Design review of the part built by this model. Coordinates are the model's own, in mm. Face numbers are marked on the shaded views. A direction names the side the tool comes from. Round coordinates to 2 decimals unless told otherwise and drop trailing zeros. Loops run counter-clockwise (first coordinate to the right, second up) from the corner with the lowest first, then second, coordinate; pieces in that order, holes last. Notation, with made-up numbers: (0.25, 60) - (16.25, 60) arc R12 cw to (16.25, 72) - close; hole circle Ø6 at (44.25, 70.5). An arc over 180 degrees is marked (long way). Answer as CSV lines item,"result". Start each with the question number.
(1) Consider section C-C (z = 13). Give the boundary of the cut face in (x, y), and give its area (3 significant figures).
(2) For P1, Ø6, axis at x = 45, z = 5.5, coming from the -Y side; P2, Ø12, axis at y = 23, z = -12.5, coming from the -X side; P3, Ø2, axis at y = 10, z = 1, coming from the +X side, all flat-tipped, find the tip position at first contact; note any pin that passes through.
(3) Consider section D-D (y = 25.5). Give the boundary of the cut face in (x, z), and give its area (3 significant figures).
(4) Consider section A-A (y = 18.75). Give the boundary of the cut face in (x, z).
(5) Consider section B-B (y = 5). Give the boundary of the cut face in (x, z).
(6) Mouldability with a two-part tool opening along X and no side actions: class the marked faces 6, 7 and 8 as released by +X, released by -X, zero draft, split by the parting line, or undercut.
(7) Wall thickness on L1, parallel to Z at x = 61, y = 24; L2, parallel to Y at x = 32, z = -8.5; L3, parallel to Y at x = -2, z = 12.5: over which ranges is each line inside the solid? List them lowest first.
(8) For the marked faces 1, 2, 3, 4 and 5, list the 3-axis set-ups (+Z, -Z, +X, -X, +Y, -Y) from which the entire face can be reached by the end or side of a thin tool; tool diameter is ignored.
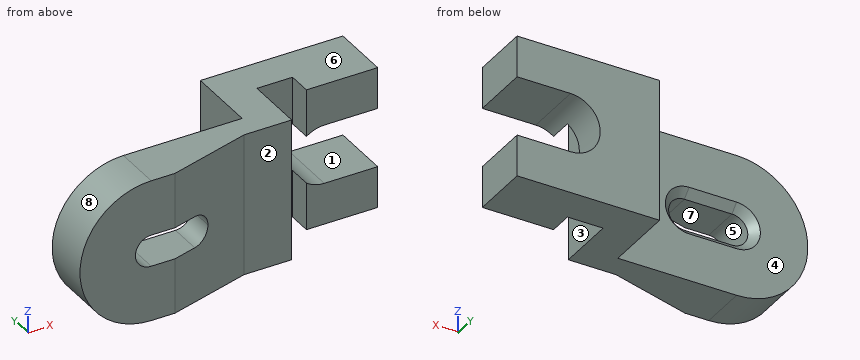
from build123d import *

# Parameters (mm, degrees)
HUB_SKETCH_R                = 18
HUB_36_DEPTH                = 12
ARM_START                   = -12
ARM_DEPTH                   = 12
HUB_SLOT_CHAMFER_45_DEPTH   = 2
HUB_SLOT_CHAMFER_45_DRAFT   = -45
HUB_SLOT_DEPTH              = 18
CLEVIS_BLOCK_DEPTH          = 36
CLEVIS_U_SLOT_SKETCH_W      = 13.5
CLEVIS_U_SLOT_SKETCH_H      = 15
CLEVIS_U_SLOT_DEPTH         = 90
BLOCK_STEP_CUT_DEPTH        = 60
BLOCK_STEP_CUT_DEPTH_BACK   = 147
BLOCK_STEP_CUT_SKETCH_W     = 9
BLOCK_STEP_CUT_SKETCH_H     = 21
ARM_TAPER_CUT_DEPTH         = 73
ARM_TAPER_CUT_DEPTH_BACK    = 190
ARM_TAPER_CUT_SKETCH_W      = 18
ARM_TAPER_CUT_SKETCH_H      = 15
BLOCK_RELIEF_CUT_DEPTH      = 190
BLOCK_RELIEF_CUT_DEPTH_BACK = 190


with BuildPart() as part:
    # Hub Sketch → Hub _36 (new body)
    with BuildSketch(Plane(origin=(0, 0, 0), x_dir=(1, 0, 0), z_dir=(0, 1, 0))):
        with Locations(Location((0, 0, 0), (0, 0, 270))):
            Circle(HUB_SKETCH_R)
    extrude(amount=HUB_36_DEPTH)

    # Arm Sketch → Arm (add)
    with BuildSketch(Plane(origin=(0, 12, 0), x_dir=(1, 0, 0), z_dir=(0, 1, 0)).offset(ARM_START)):
        with BuildLine():
            Line((30, 0), (18, 0))
            ThreePointArc((18, 0), (12.727922061, -12.727922061), (0, -18))
            Line((0, -18), (30, -18))
            Line((30, -18), (30, 0))
        make_face()
        with BuildLine():
            ThreePointArc((0, 18), (12.727922061, 12.727922061), (18, 0))
            Line((18, 0), (30, 0))
            Line((30, 0), (30, 18))
            Line((30, 18), (0, 18))
        make_face()
    extrude(amount=ARM_DEPTH)


with BuildPart() as hub_slot_chamfer_45_tool:
    # Hub Slot Chamfer Sketch → Hub Slot Chamfer 45 (with draft: the straight prism first)
    with BuildSketch(Plane(origin=(0, 12, 0), x_dir=(1, 0, 0), z_dir=(0, 1, 0))):
        with BuildLine():
            ThreePointArc((0, 6), (-6, 0), (0, -6))
            Line((0, -6), (12, -6))
            ThreePointArc((12, -6), (18, 0), (12, 6))
            Line((12, 6), (0, 6))
        make_face()
    extrude(amount=-HUB_SLOT_CHAMFER_45_DEPTH)
    # Hub Slot Chamfer 45: the draft: its side faces are tilted about the plane it starts from
    hub_slot_chamfer_45_sides = [hub_slot_chamfer_45_tool.faces().sort_by_distance(p)[0] for p in [
        (6, 11, -6),
        (-6, 11, 0),
        (6, 11, 6),
        (18, 11, 0),
    ]]
    draft(hub_slot_chamfer_45_sides, Plane(origin=(0, 12, 0), x_dir=(1, 0, 0), z_dir=(0, 1, 0)), HUB_SLOT_CHAMFER_45_DRAFT)


with BuildPart() as part_1:
    add(part.part)

    # Hub Slot Chamfer 45: cut by hub_slot_chamfer_45_tool
    add(hub_slot_chamfer_45_tool.part, mode=Mode.SUBTRACT)

    # Hub Slot Sketch → Hub Slot (cut)
    with BuildSketch(Plane(origin=(0, 10, 0), x_dir=(1, 0, 0), z_dir=(0, 1, 0))):
        with BuildLine():
            Line((12, 4), (0, 4))
            ThreePointArc((0, 4), (2.828427125, 2.828427125), (4, 0))
            ThreePointArc((4, 0), (2.828427125, -2.828427125), (0, -4))
            Line((0, -4), (12, -4))
            ThreePointArc((12, -4), (8, 0), (12, 4))
        make_face()
        with BuildLine():
            ThreePointArc((4, 0), (2.828427125, 2.828427125), (0, 4))
            ThreePointArc((0, 4), (-4, 0), (0, -4))
            ThreePointArc((0, -4), (2.828427125, -2.828427125), (4, 0))
        make_face()
        with BuildLine():
            ThreePointArc((16, 0), (14.828427125, 2.828427125), (12, 4))
            ThreePointArc((12, 4), (8, 0), (12, -4))
            ThreePointArc((12, -4), (14.828427125, -2.828427125), (16, 0))
        make_face()
    extrude(amount=-HUB_SLOT_DEPTH, mode=Mode.SUBTRACT)

    # Clevis Block Sketch → Clevis Block (add)
    with BuildSketch(Plane.XY.offset(18)):
        Polygon((30, 12), (30, 30), (66, 30), (66, 15), (66, 0), (30, 0), align=None)
    extrude(amount=-CLEVIS_BLOCK_DEPTH)

    # Clevis U-Slot Sketch → Clevis U-Slot (cut)
    with BuildSketch(Plane(origin=(0, 30, 0), x_dir=(1, 0, 0), z_dir=(0, 1, 0))):
        with BuildLine():
            Line((52.5, -7.5), (52.5, 7.5))
            ThreePointArc((52.5, 7.5), (45, 0), (52.5, -7.5))
        make_face()
        with Locations((59.25, 0)):
            Rectangle(CLEVIS_U_SLOT_SKETCH_W, CLEVIS_U_SLOT_SKETCH_H)
    extrude(amount=-CLEVIS_U_SLOT_DEPTH, mode=Mode.SUBTRACT)

    # Block Step Cut Sketch → Block Step Cut (cut, two sides: drawn at the far end of the back side and taken through both)
    with BuildSketch(Plane.XY.offset(18).offset(-BLOCK_STEP_CUT_DEPTH_BACK)):
        with Locations((43.5, 10.5)):
            Rectangle(BLOCK_STEP_CUT_SKETCH_W, BLOCK_STEP_CUT_SKETCH_H)
    extrude(amount=BLOCK_STEP_CUT_DEPTH + BLOCK_STEP_CUT_DEPTH_BACK, mode=Mode.SUBTRACT)

    # Arm Taper Cut Sketch → Arm Taper Cut (cut, two sides: drawn at the far end of the back side and taken through both)
    with BuildSketch(Plane.XY.offset(18).offset(-ARM_TAPER_CUT_DEPTH_BACK)):
        with Locations((57, 7.5)):
            Rectangle(ARM_TAPER_CUT_SKETCH_W, ARM_TAPER_CUT_SKETCH_H)
    extrude(amount=ARM_TAPER_CUT_DEPTH + ARM_TAPER_CUT_DEPTH_BACK, mode=Mode.SUBTRACT)

    # Block Relief Cut Sketch → Block Relief Cut (cut, two sides: drawn at the far end of the back side and taken through both)
    with BuildSketch(Plane.XY.offset(18).offset(-BLOCK_RELIEF_CUT_DEPTH_BACK)):
        Polygon((39, 0), (39, 6), (27, 6), (6, 0), align=None)
    extrude(amount=BLOCK_RELIEF_CUT_DEPTH + BLOCK_RELIEF_CUT_DEPTH_BACK, mode=Mode.SUBTRACT)


solid = part_1.part
Determined:
1,outline,"(-12.45, 0) - (6, 0) - (27, 6) - (39, 6) - (39, 21) - (48, 21) - (48, 15) - (66, 15) - (66, 30) - (30, 30) - (30, 12) - (-12.45, 12) - close"
1,area,"995 mm^2"
2,P1,"stops at y = 21"
2,P2,"stops at x = 30"
2,P3,"stops at x = 39"
3,outline,"(30, -18) - (66, -18) - (66, -7.5) - (52.5, -7.5) arc R7.5 cw to (52.5, 7.5) - (66, 7.5) - (66, 18) - (30, 18) - close"
3,area,"1,010 mm^2"
4,outline,"(30, -18) - (39, -18) - (39, 18) - (30, 18) - close; (48, -18) - (66, -18) - (66, -7.5) - (52.5, -7.5) arc R7.5 cw to (48, -6) - close; (48, 6) arc R7.5 cw to (52.5, 7.5) - (66, 7.5) - (66, 18) - (48, 18) - close"
5,outline,"(0, -18) - (23.5, -18) - (23.5, 18) - (0, 18) arc R18 ccw to start; hole (0, -4) - (12, -4) arc R4 ccw to (12, 4) - (0, 4) arc R4 ccw to start"
6,face 6,"zero draft"
6,face 7,"undercut"
6,face 8,"released by -X"
7,L1,"z = -18 to -7.5, 7.5 to 18"
7,L2,"y = 6 to 30"
7,L3,"y = 0 to 12"
8,face 1,"+X, +Y, -Y"
8,face 2,"+Z, -Z, +X, -Y"
8,face 3,"+Z, -Z, -Y"
8,face 4,"+Z, -Z, -X, +Y"
8,face 5,"+Y, -Y"
